For this review, take the finished solid that the model builds, in its own axes (mm). Face numbers are marked on the shaded views. Coordinates: 2 decimals unless noted, no trailing zeros. Loops run counter-clockwise (first coordinate to the right, second up) from the corner with the lowest first, then second, coordinate; pieces in that order, holes last. Notation, with made-up numbers: M 27,41 L 33,41 A24 ccw 33,67 Z; hole C -24.5,-19.5 d9. An arc over 180 degrees is marked long. Answer as a JSON object with one key per item and string values. Group by question number.
Item 1: Add section A-A (z = 0). State the section outline as (x, y) points.
Item 2: Add section C-C (y = -33). State the section outline as (x, z) points.
Item 3: Wall thickness on L1, parallel to X at y = -5, z = 0; L2, parallel to X at y = 6, z = -26; L3, parallel to Z at x = 83, y = -41.5: over which ranges is each line inside the solid? List them lowest first. Write a range as from..to.
Item 4: Mouldability with a two-part tool opening along Z and no side actions: class the marked faces 1, 2, 3 and 4 as +Z half, -Z half, draft (parallel to the pull), parting line (faces both ways), or undercut.
Item 5: Add section B-B (x = -64.5). State the section outline as (y, z) points.
Item 6: Add section D-D (x = 60). State the section outline as (y, z) points, then the cut area to 3 significant figures.
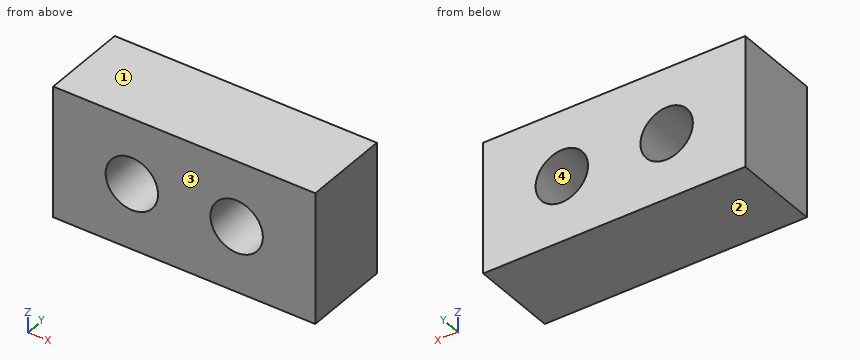
from build123d import *

# Parameters (mm, degrees)
SKETCH1_W           = 300
SKETCH1_H           = 150
SKETCH1_R           = 30
BOSS_EXTRUDE1_DEPTH = 50


with BuildPart() as part:
    # Sketch1 → Boss-Extrude1 (new, symmetric)
    with BuildSketch(Plane(origin=(0, 0, 0), x_dir=(1, 0, 0), z_dir=(0, 1, 0))):
        Rectangle(SKETCH1_W, SKETCH1_H)
        with Locations(Location((60, 0, 0), (0, 0, 90))):
            Circle(SKETCH1_R, mode=Mode.SUBTRACT)
        with Locations(Location((-60, 0, 0), (0, 0, 90))):
            Circle(SKETCH1_R, mode=Mode.SUBTRACT)
    extrude(amount=BOSS_EXTRUDE1_DEPTH, both=True)


solid = part.part
From the geometry:
{
 "1": {"outline": "M -150,-50 L -90,-50 L -90,50 L -150,50 Z; M -30,-50 L 30,-50 L 30,50 L -30,50 Z; M 90,-50 L 150,-50 L 150,50 L 90,50 Z"},
 "2": {"outline": "M -150,-75 L 150,-75 L 150,75 L -150,75 Z; hole C -60,0 d60; hole C 60,0 d60"},
 "3": {"L1": "x = -150..-90, -30..30, 90..150", "L2": "x = -150..-74.97, -45.03..45.03, 74.97..150", "L3": "z = -75..-19.26, 19.26..75"},
 "4": {"face 1": "+Z half", "face 2": "-Z half", "face 3": "draft", "face 4": "undercut"},
 "5": {"outline": "M -50,-75 L 50,-75 L 50,-29.66 L -50,-29.66 Z; M -50,29.66 L 50,29.66 L 50,75 L -50,75 Z"},
 "6": {"outline": "M -50,-75 L 50,-75 L 50,-30 L -50,-30 Z; M -50,30 L 50,30 L 50,75 L -50,75 Z", "area": "9,000 mm²"}
}
